Build history of the part. All positions in model axes, mm. Give positions to 0.01 mm unless a question says otherwise; leave off trailing zeros. Loops run counter-clockwise (first coordinate to the right, second up) from the corner with the lowest first, then second, coordinate; pieces in that order, holes last. Notation, with made-up numbers: M -2.75,1.5 L 47.25,1.5 A16 cw 47.25,19.5 Z; hole C -15.5,54 d10. An arc over 180 degrees is marked long. Put each result on its own line as item: value.
```python
from build123d import *

# Parameters (mm, degrees)
SKETCH1_W           = 96
SKETCH1_H           = 32
BOSS_EXTRUDE1_DEPTH = 6
FILLET1_R           = 5
SKETCH2_R           = 5.5
CUT_EXTRUDE1_DEPTH  = 6
LPATTERN1_COUNT     = 2
LPATTERN1_PITCH     = 60


with BuildPart() as part:
    # Sketch1 → Boss-Extrude1 (new body)
    with BuildSketch(Plane.XY):
        with Locations((48, -16)):
            Rectangle(SKETCH1_W, SKETCH1_H)
    extrude(amount=BOSS_EXTRUDE1_DEPTH)

    # Fillet1
    fillet1_edges = [part.edges().sort_by_distance(p)[0] for p in [
        (0, 0, 3),
        (96, 0, 3),
        (96, -32, 3),
        (0, -32, 3),
    ]]
    fillet(fillet1_edges, radius=FILLET1_R)

    # Sketch2 → Cut-Extrude1 (cut)
    with BuildSketch(Plane.XY.offset(6)):
        with Locations((18, -16)):
            Circle(SKETCH2_R)
    cut_extrude1 = extrude(amount=-CUT_EXTRUDE1_DEPTH, mode=Mode.SUBTRACT)

    # LPattern1: Cut-Extrude1 ×2
    with Locations(*[(i * LPATTERN1_PITCH, 0, 0) for i in range(1, LPATTERN1_COUNT)]):
        add(cut_extrude1, mode=Mode.SUBTRACT)


solid = part.part
```
Q1. Slice it at B-B (z = 3.85). List the corners of the cut face in (x, y), and give its area (3 significant figures).
Here are the results:
outline: M 0,-27 A5 ccw 5,-32 L 91,-32 A5 ccw 96,-27 L 96,-5 A5 ccw 91,0 L 5,0 A5 ccw 0,-5 Z; hole C 18,-16 d11; hole C 78,-16 d11
area: 2,860 mm²
Q2. Slice it at A-A (x = 18). List the corners of the cut face in (y, z), and give its area (3 significant figures).
Here are the results:
outline: M -32,0 L -21.5,0 L -21.5,6 L -32,6 Z; M -10.5,0 L 0,0 L 0,6 L -10.5,6 Z
area: 126 mm²
Q3. Probe line 1 (Y direction, x = 78, z = 4.7); line 2 (X direction, y = -20, z = 3.6); line 3 (Y direction, x = 81.5, z = 1.8). List the from-to ranges inside material, lowest first. Write a range as from..to.
Here are the results:
line 1: -32..-21.5, -10.5..0
line 2: 0..14.23, 21.77..74.23, 81.77..96
line 3: -32..-20.24, -11.76..0
Q4. Mould opens along Y. For faces 1 (the flat face through (96, -16, 3)), 2 (the cylindrical face through (1, -30, 3)), 3 (the cylindrical face through (16.81, -21.37, 3.04)) say: pulls with the +Y half, pulls with the -Y half, needs draft (parallel to the pull), parting line crosses it, or undercut.
Here are the results:
face 1: needs draft
face 2: pulls with the -Y half
face 3: undercut
Q5. Slice it at C-C (y = -16). List the corners of the cut face in (x, z).
Here are the results:
outline: M 0,0 L 12.5,0 L 12.5,6 L 0,6 Z; M 23.5,0 L 72.5,0 L 72.5,6 L 23.5,6 Z; M 83.5,0 L 96,0 L 96,6 L 83.5,6 Z
